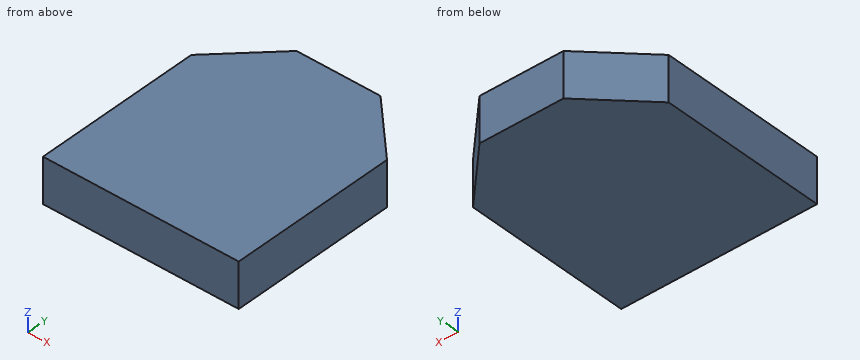
from build123d import *

# Parameters (mm, degrees)
BOSS_EXTRUDE1_DEPTH = 8


with BuildPart() as part:
    # Sketch1 → Boss-Extrude1 (new body)
    with BuildSketch(Plane.XY):
        Polygon((0, 30), (10, 40), (25, 40), (35, 30), (35, 0), (0, 0), align=None)
    extrude(amount=BOSS_EXTRUDE1_DEPTH)


solid = part.part
Model file for the job. Use its own axes, mm. Give positions to 0.01 mm unless a question says otherwise; leave off trailing zeros. Order: outer loops, then holes, each group sorted by start corner. A loop starts at its lowest first (then second) coordinate and runs counter-clockwise, first axis right, second up. Notation, with made-up numbers: (-6, -6) - (35, -6) arc R26 ccw to (35, 21) - close; hole circle Ø6 at (15.25, -0.75). An arc over 180 degrees is marked (long way). Write item = value, one per line. Start each with the question number.
1. Cut at B-B, the plane y = 37.5. List the corners of the cut face in (x, z).
2. Probe line 1 along Y through (x, z) = (25.5, 4.25); line 2 along Y through (x, z) = (28, 3.5). List the from-to ranges inside material, lowest first.
3. Cut at C-C, the plane x = 27. List the corners of the cut face in (y, z), and give its area (3 significant figures).
4. Cut at A-A, the plane z = 0.5. List the corners of the cut face in (x, y), and give its area (3 significant figures).
Taken from the geometry:
q1.outline = (7.5, 0) - (27.5, 0) - (27.5, 8) - (7.5, 8) - close
q2.line_1 = 0 to 39.5
q2.line_2 = 0 to 37
q3.outline = (0, 0) - (38, 0) - (38, 8) - (0, 8) - close
q3.area = 304 mm²
q4.outline = (0, 0) - (35, 0) - (35, 30) - (25, 40) - (10, 40) - (0, 30) - close
q4.area = 1,300 mm²
